```python
from build123d import *

# Parameters (mm, degrees)
SKETCH_1_W               = 100
SKETCH_1_H               = 335
EXTRUDE_1_DEPTH          = 35
CHAMFER_1_SIZE           = 20
CUT_EXTRUDE_1_DEPTH      = 179.27296486
CUT_EXTRUDE_1_DEPTH_BACK = 179.27296486
SKETCH_2_R               = 11


with BuildPart() as part:
    # 草图1 → 凸台-拉伸1 (new body)
    with BuildSketch(Plane.XY):
        Rectangle(SKETCH_1_W, SKETCH_1_H)
    extrude(amount=EXTRUDE_1_DEPTH)

    # 倒角1
    chamfer_1_edges = [part.edges().sort_by_distance(p)[0] for p in [
        (50, 167.5, 17.5),
    ]]
    chamfer(chamfer_1_edges, length=CHAMFER_1_SIZE)

    # 草图2 → 切除-拉伸1 (cut, two sides: drawn at the far end of the back side and taken through both)
    with BuildSketch(Plane.XY.offset(35).offset(-CUT_EXTRUDE_1_DEPTH_BACK)):
        with Locations((10, 141.327613457)):
            Circle(SKETCH_2_R)
        with Locations((10, -118.672386543)):
            Circle(SKETCH_2_R)
        with Locations((10, 11.327613457)):
            Circle(SKETCH_2_R)
    extrude(amount=CUT_EXTRUDE_1_DEPTH + CUT_EXTRUDE_1_DEPTH_BACK, mode=Mode.SUBTRACT)


solid = part.part
```
Read the model definition and answer for the solid it produces. Units are mm, in the model's axes. Coordinates: 2 decimals unless noted, no trailing zeros. Loops run counter-clockwise (first coordinate to the right, second up) from the corner with the lowest first, then second, coordinate; pieces in that order, holes last.
(1) The part is cut by section C-C (x = 43.5). Determine the outline of the cut face in (y, z).
Solution:
outline: (-167.5, 0) - (154, 0) - (154, 35) - (-167.5, 35) - close
(2) The part is cut by section A-A (x = 10). Determine the outline of the cut face in (y, z).
Solution:
outline: (-167.5, 0) - (-129.67, 0) - (-129.67, 35) - (-167.5, 35) - close; (-107.67, 0) - (0.33, 0) - (0.33, 35) - (-107.67, 35) - close; (22.33, 0) - (130.33, 0) - (130.33, 35) - (22.33, 35) - close; (152.33, 0) - (167.5, 0) - (167.5, 35) - (152.33, 35) - close
(3) The mould has two halves that part along Y. Classify faces 1 (the face through (50, -12, 17)), 2 (the face through (20.5, 14.6, 17.3)), 3 (the face through (-11, 167.5, 17)), 4 (the face through (8.568, 152.234, 17.255)): released by +Y, released by -Y, zero draft, split by the parting line, or undercut.
Solution:
face 1: zero draft
face 2: undercut
face 3: released by +Y
face 4: undercut
(4) The part is cut by section B-B (z = 19.5). Determine the outline of the cut face in (x, y), and give its area (3 significant figures).
Solution:
outline: (-50, -167.5) - (50, -167.5) - (50, 147.5) - (30, 167.5) - (-50, 167.5) - close; hole circle Ø22 at (10, -118.67); hole circle Ø22 at (10, 11.33); hole circle Ø22 at (10, 141.33)
area: 32,200 mm2
(5) Consider line 1 along Y through (x, z) = (10, 18.5); line 2 along X through (y, z) = (10.5, 10.5); line 3 along Y through (x, z) = (11, 16). Determine where each line is inside the solid, lowest interval first.
Solution:
line 1: y = -167.5 to -129.67, -107.67 to 0.33, 22.33 to 130.33, 152.33 to 167.5
line 2: x = -50 to -0.97, 20.97 to 50
line 3: y = -167.5 to -129.63, -107.72 to 0.37, 22.28 to 130.37, 152.28 to 167.5
